from build123d import *

# Parameters (mm, degrees)
SKETCH1_W          = 20
SKETCH1_H          = 165
SKETCH1_W_2        = 32.5
SKETCH1_H_2        = 50
SKETCH1_W_3        = 12.5
SKETCH1_H_3        = 10
SKETCH6_R          = 6
CUT_EXTRUDE1_DEPTH = 80


with BuildPart() as part:
    # Sketch1 → Revolve7 (revolve)
    with BuildSketch(Plane.XY, mode=Mode.PRIVATE) as revolve7_sk:
        with Locations((10, -108.875)):
            Rectangle(SKETCH1_W, SKETCH1_H)
        Polygon((0, -26.375), (23.5, -26.375), (32.5, -17.375), (0, -17.375), align=None)
        with Locations((16.25, 7.625)):
            Rectangle(SKETCH1_W_2, SKETCH1_H_2)
        Polygon((0, 32.625), (0, 41.625), (23.5, 41.625), (32.5, 32.625), align=None)
        with Locations((6.25, 46.625)):
            Rectangle(SKETCH1_W_3, SKETCH1_H_3)
    revolve(revolve7_sk.sketch.rotate(Axis((0, -26.375, 0), (0, -1, 0)), 180), axis=Axis((0, -26.375, 0), (0, -1, 0)))

    # Sketch5 → Cut-Revolve1 (revolve, cut)
    with BuildSketch(Plane.XY, mode=Mode.PRIVATE) as cut_revolve1_sk:
        Polygon((0, 51.625), (0, 24.625), (0, 21.625), (6, 24.625), (6, 51.625), align=None)
    revolve(cut_revolve1_sk.sketch.rotate(Axis((0, 51.625, 0), (0, -1, 0)), 180), axis=Axis((0, 51.625, 0), (0, -1, 0)), mode=Mode.SUBTRACT)

    # Sketch6 → Cut-Extrude1 (cut, symmetric)
    with BuildSketch(Plane.XY):
        with Locations((0, 7.625)):
            Circle(SKETCH6_R)
    extrude(amount=CUT_EXTRUDE1_DEPTH, both=True, mode=Mode.SUBTRACT)


solid = part.part
The model under review builds one solid part; all positions refer to its coordinate system, in mm. A direction names the side the tool comes from. Round coordinates to 2 decimals unless told otherwise and drop trailing zeros. Order: outer loops, then holes, each group sorted by start corner. A loop starts at its lowest first (then second) coordinate and runs counter-clockwise, first axis right, second up. Notation, with made-up numbers: (-22.75, 42.5) -> (-3.75, 42.5) arc R22 ccw to (-3.75, 64.5) -> close; hole circle Ø11 at (-37.5, 11). An arc over 180 degrees is marked (long way). Use CSV: the item, a comma, the result in double quotes. Start each with the question number.
(1) Consider section A-A on y = -40.5. Write out the cut boundary in (x, z), and give its area (3 significant figures).
(2) Insertion check: pin 1 (8 mm diameter, centred on x = -21.5, y = -71, fed in from -Z); pin 2 (5 mm diameter, centred on x = -2.5, y = -90, fed in from -Z); pin 3 (1.5 mm diameter, centred on x = 14.5, z = 25.5, fed in from -Y); pin 4 (11 mm diameter, centred on x = 0, y = 7.625, fed in from -Z) (3 decimals). Each pin has a flat end and moves straight along its axis. Give the tip position at first contact, or say it passes through.
(3) Wall thickness on probe 1 along Z at (x, y) = (0, 46); probe 2 along Y at (x, z) = (0, -11) (3 decimals); probe 3 along Z at (x, y) = (-1, -142): over which ranges is each line inside the solid? List them lowest first. Write a range as from..to.
(4) Mouldability with a two-part tool opening along X and no side actions: class faces 4 (the face through (0, -191.375, 0)), 5 (the face through (0.081, 21.813, 0.366)), 6 (the face through (-1.301, 1.768, 0.455)), 7 (the face through (7.045, 7.975, 31.727)) as pulls with the +X half, pulls with the -X half, needs draft (parallel to the pull), parting line crosses it, or undercut.
(5) Tool access review of faces 1 (the face through (10, 41.625, 10)), 2 (the face through (19.98, -107.72, -0.88)), 3 (the face through (-3, 51.625, 5.4)): name each direction out of +Z, -Z, +X, -X, +Y, -Y from which nothing blocks a thin tool from reaching the whole face with its end or side.
(6) Consider section B-B on y = 11. Write out the cut boundary in (x, z).
Responses:
1,outline,"circle Ø40 at (0, 0)"
1,area,"1,260 mm²"
2,pin 1,"z = -9.68"
2,pin 2,"z = -20"
2,pin 3,"y = -21.29"
2,pin 4,"through"
3,probe 1,"-12.5..-6, 6..12.5"
3,probe 2,"-191.375..1.625, 13.625..51.625"
3,probe 3,"-19.97..19.97"
4,face 4,"needs draft"
4,face 5,"undercut"
4,face 6,"undercut"
4,face 7,"parting line crosses it"
5,face 1,"+Y"
5,face 2,"-Y"
5,face 3,"+Z, -Z, +X, -X, +Y"
6,outline,"(-4.96, -32.12) -> (-4.96, 32.12) arc R32.5 ccw to start; (4.96, -32.12) arc R32.5 ccw to (4.96, 32.12) -> close"
